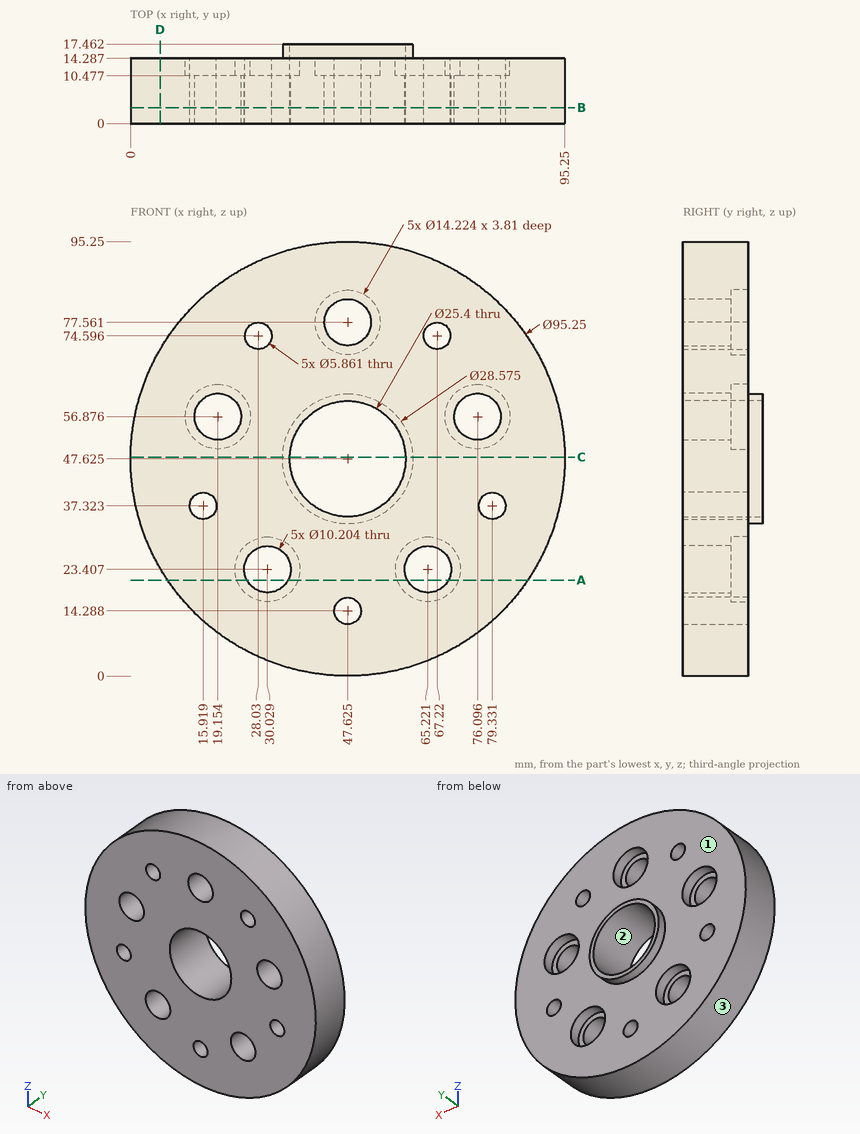
Answer from the drawing. Dimensions are ordinates in mm from the lowest x, y and z of the part. Give positions to 0.01 mm unless a question says otherwise; leave off trailing zeros. Order: outer loops, then holes, each group sorted by start corner. A loop starts at its lowest first (then second) coordinate and runs counter-clockwise, first axis right, second up. Notation, with made-up numbers: (49, 58.25) -> (78, 58.25) arc R24 cw to (78, 73.25) -> close; hole circle Ø3 at (68.25, 83.25). An arc over 180 degrees is marked (long way). Answer as a JSON object with one key per item and string values. Group by question number.
1. Section A-A on z = 21 is taken. Determine the outline of the cut face in (x, y).
2. Section C-C on z = 48 is taken. Determine the outline of the cut face in (x, y), plus the area to 3 significant figures.
3. The mould has two halves that part along X. Classify the marked faces 1, 2 and 3: released by +X, released by -X, zero draft, split by the parting line, or undercut.
4. Section D-D on x = 6.5 is taken. Determine the outline of the cut face in (y, z).
5. Section B-B on y = 3.5 is taken. Count the separate pieces of the cut face and the enclosed holes in it.
6. Flat-ended cylindrical pins translate along their axes: pin 1 Ø13.5 at (x, z) = (76.1, 56.88) entering from +Y; pin 2 Ø2 at (y, z) = (12, 58.5) entering from -X (1 decimal); pin 3 Ø10 at (x, y) = (73.5, 3.5) entering from -Z. Find the tip coordinate at first contact, or state that the pin passes through.
7. Consider line 1 along Z through (x, y) = (65.5, 1.25) (1 decimal); line 2 along Z through (x, y) = (47.5, 15.5) (1 decimal); line 3 along X through (y, z) = (7, 58.5) (1 decimal). Determine where each line is inside the solid, lowest interval first. Write a range as [from, to].
Result sheet:
{
 "1": {"outline": "(8.14, 0) -> (25.53, 0) -> (25.53, 10.48) -> (23.34, 10.48) -> (23.34, 14.29) -> (8.14, 14.29) -> close; (34.53, 0) -> (60.72, 0) -> (60.72, 10.48) -> (58.53, 10.48) -> (58.53, 14.29) -> (36.72, 14.29) -> (36.72, 10.48) -> (34.53, 10.48) -> close; (69.72, 0) -> (87.11, 0) -> (87.11, 14.29) -> (71.91, 14.29) -> (71.91, 10.48) -> (69.72, 10.48) -> close"},
 "2": {"outline": "(0, 0) -> (34.93, 0) -> (34.93, 17.46) -> (33.34, 17.46) -> (33.34, 14.29) -> (0, 14.29) -> close; (60.32, 0) -> (95.25, 0) -> (95.25, 14.29) -> (61.91, 14.29) -> (61.91, 17.46) -> (60.32, 17.46) -> close", "area": "1,010 mm^2"},
 "3": {"face 1": "zero draft", "face 2": "undercut", "face 3": "split by the parting line"},
 "4": {"outline": "(0, 23.61) -> (14.29, 23.61) -> (14.29, 71.64) -> (0, 71.64) -> close"},
 "5": {"separate pieces": "1", "enclosed holes": "11"},
 "6": {"pin 1": "stops at y = 10.48", "pin 2": "stops at x = 1", "pin 3": "stops at z = 4.82"},
 "7": {"line 1": "z = [3.5, 18.3], [28.5, 72.2], [77, 91.8]", "line 2": "z = [33.3, 34.9], [60.3, 61.9]", "line 3": "x = [1.3, 14.3], [24, 41.1], [54.2, 71.3], [80.9, 94]"}
}
